```python
from build123d import *

# Parameters (mm, degrees)
SKETCH1_R           = 20
BOSS_EXTRUDE1_DEPTH = 8


with BuildPart() as part:
    # Sketch1 → Boss-Extrude1 (new body)
    with BuildSketch(Plane.XY):
        with BuildLine():
            Line((0, 0), (110, 0))
            Line((110, 0), (110, 55))
            ThreePointArc((110, 55), (96.819805153, 86.819805153), (65, 100))
            Line((65, 100), (0, 100))
            Line((0, 100), (0, 0))
        make_face()
        with Locations((65, 55)):
            Circle(SKETCH1_R, mode=Mode.SUBTRACT)
    extrude(amount=BOSS_EXTRUDE1_DEPTH)


solid = part.part
```
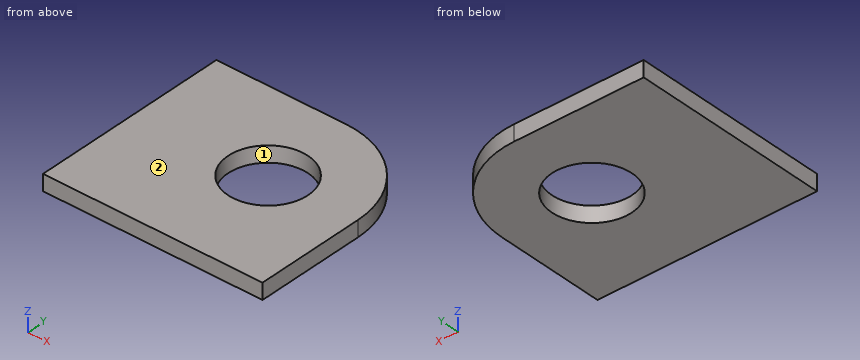
Build history of the part. All positions in model axes, mm. Face numbers are marked on the shaded views. Round coordinates to 2 decimals unless told otherwise and drop trailing zeros. Write each loop counter-clockwise with the first axis right and the second up, starting at its lowest first coordinate (ties: lowest second). Pieces come first, ordered by that corner, then holes.
1) Band-saw the part on B-B, the plane x = 50. List the corners of the cut face in (y, z), and give its area (3 significant figures).
2) Band-saw the part on D-D, the plane x = 102. List the corners of the cut face in (y, z), and give its area (3 significant figures).
3) Band-saw the part on C-C, the plane y = 90. List the corners of the cut face in (x, z).
4) Band-saw the part on A-A, the plane z = 5.25. List the corners of the cut face in (x, y).
5) Mould opens along X. For the marked faces 1 and 2 say: +X half, -X half, draft (parallel to the pull), parting line (faces both ways), or undercut.
6) Drill centre lines: probe 1 along Y at (x, z) = (65, 3.5); probe 2 along X at (y, z) = (54, 5.75); probe 3 along X at (y, z) = (62, 2.75) (3 decimals). Where is each one in solid material? Low to high.
Ans:
1. outline: (0, 0) - (41.77, 0) - (41.77, 8) - (0, 8) - close; (68.23, 0) - (100, 0) - (100, 8) - (68.23, 8) - close
1. area: 588 mm2
2. outline: (0, 0) - (80.61, 0) - (80.61, 8) - (0, 8) - close
2. area: 645 mm2
3. outline: (0, 0) - (93.28, 0) - (93.28, 8) - (0, 8) - close
4. outline: (0, 0) - (110, 0) - (110, 55) arc R45 ccw to (65, 100) - (0, 100) - close; hole circle Ø40 at (65, 55)
5. face 1: undercut
5. face 2: draft
6. probe 1: y = 0 to 35, 75 to 100
6. probe 2: x = 0 to 45.03, 84.97 to 110
6. probe 3: x = 0 to 46.265, 83.735 to 109.452
